Read the model definition and answer for the solid it produces. Units are mm, in the model's axes. Face numbers are marked on the shaded views. Round coordinates to 2 decimals unless told otherwise and drop trailing zeros. Order: outer loops, then holes, each group sorted by start corner. A loop starts at its lowest first (then second) coordinate and runs counter-clockwise, first axis right, second up. Notation, with made-up numbers: (58.5, -10.75) -> (90.5, -10.75) arc R25 cw to (90.5, 26.25) -> close; hole circle Ø1 at (28, 8). An arc over 180 degrees is marked (long way). Answer as a JSON object with one key per item and string values. Group by question number.
Item 1: Given P1, Ø6.5, axis at x = -44, z = -1.5, coming from the +Y side; P2, Ø2, axis at x = -4, z = -8, coming from the +Y side; P3, Ø2, axis at y = -2, z = -8.5, coming from the +X side; P4, Ø4.5, axis at x = -45.5, z = 0, coming from the +Y side, each flat-ended and moving along its own axis, determine where each tip first touches the part or whether it passes through.
Item 2: Section A-A, the plane z = 0 is taken. Count the separate pieces of the cut face and the enclosed holes in it, plus the area to 3 significant figures.
Item 3: Section C-C, the plane z = 10 is taken. Write down the section's boundary in (x, y), plus the area to 3 significant figures.
Item 4: Consider probe 1 along X at (y, z) = (-1.15, 0); probe 2 along Z at (x, y) = (32.5, 1.1); probe 3 along X at (y, z) = (-2.05, 1). Determine where each line is inside the solid, lowest interval first. Write a range as from..to.
Item 5: Section B-B, the plane x = -32 is taken. Write down the section's boundary in (y, z), plus the area to 3 significant figures.
Item 6: The mould has two halves that part along Z. Classify the marked faces 1 and 2: pulls with the +Z half, pulls with the -Z half, needs draft (parallel to the pull), parting line crosses it, or undercut.
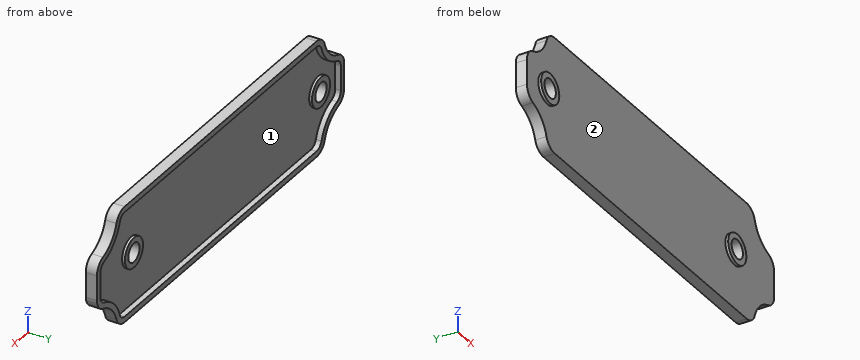
from build123d import *

# Parameters (mm, degrees)
BASE_PLATE_DEPTH                = 1.5
TOP_RECESS_1_5MM_DEPTH          = 1.5
MOUNTING_HOLE_BOSSES_DEPTH      = 0.75
MOUNTING_HOLE_BOSSES_DEPTH_BACK = 2.25
HOLE_BOSS_SKETCH_R              = 4
HOLE_BOSS_SKETCH_R_2            = 2.5
MOUNTING_HOLE_SKETCH_R          = 2.5
MOUNTING_HOLES_2X_DEPTH         = 30.75


with BuildPart() as part:
    # Plate Outline Sketch → Base Plate (new, symmetric)
    with BuildSketch(Plane(origin=(0, 0, 0), x_dir=(1, 0, 0), z_dir=(0, 1, 0))):
        with BuildLine():
            Line((-42.313942393, 15.5), (42.313942393, 15.5))
            ThreePointArc((42.313942393, 15.5), (44.541774365, 14.76649875), (45.898076983, 12.852941176))
            ThreePointArc((45.898076983, 12.852941176), (48.136038969, 9.136038969), (51.852941176, 6.898076983))
            ThreePointArc((51.852941176, 6.898076983), (53.76649875, 5.541774365), (54.5, 3.313942393))
            Line((54.5, 3.313942393), (54.5, -3.313942393))
            ThreePointArc((54.5, -3.313942393), (53.76649875, -5.541774365), (51.852941176, -6.898076983))
            ThreePointArc((51.852941176, -6.898076983), (48.136038969, -9.136038969), (45.898076983, -12.852941176))
            ThreePointArc((45.898076983, -12.852941176), (44.541774365, -14.76649875), (42.313942393, -15.5))
            Line((42.313942393, -15.5), (-42.313942393, -15.5))
            ThreePointArc((-42.313942393, -15.5), (-44.541774365, -14.76649875), (-45.898076983, -12.852941176))
            ThreePointArc((-45.898076983, -12.852941176), (-48.136038969, -9.136038969), (-51.852941176, -6.898076983))
            ThreePointArc((-51.852941176, -6.898076983), (-53.76649875, -5.541774365), (-54.5, -3.313942393))
            Line((-54.5, -3.313942393), (-54.5, 3.313942393))
            ThreePointArc((-54.5, 3.313942393), (-53.76649875, 5.541774365), (-51.852941176, 6.898076983))
            ThreePointArc((-51.852941176, 6.898076983), (-48.136038969, 9.136038969), (-45.898076983, 12.852941176))
            ThreePointArc((-45.898076983, 12.852941176), (-44.541774365, 14.76649875), (-42.313942393, 15.5))
        make_face()
    extrude(amount=BASE_PLATE_DEPTH, both=True)

    # Recess Outline Sketch → Top Recess 1.5mm (cut)
    with BuildSketch(Plane(origin=(0, 1.5, 0), x_dir=(1, 0, 0), z_dir=(0, 1, 0))):
        with BuildLine():
            Line((42.313942393, 14), (-42.313942393, 14))
            ThreePointArc((-42.313942393, 14), (-43.650641576, 13.55989925), (-44.464423147, 12.411764706))
            ThreePointArc((-44.464423147, 12.411764706), (-47.075378798, 8.075378798), (-51.411764706, 5.464423147))
            ThreePointArc((-51.411764706, 5.464423147), (-52.55989925, 4.650641576), (-53, 3.313942393))
            Line((-53, 3.313942393), (-53, -3.313942393))
            ThreePointArc((-53, -3.313942393), (-52.55989925, -4.650641576), (-51.411764706, -5.464423147))
            ThreePointArc((-51.411764706, -5.464423147), (-47.075378798, -8.075378798), (-44.464423147, -12.411764706))
            ThreePointArc((-44.464423147, -12.411764706), (-43.650641576, -13.55989925), (-42.313942393, -14))
            Line((-42.313942393, -14), (42.313942393, -14))
            ThreePointArc((42.313942393, -14), (43.650641576, -13.55989925), (44.464423147, -12.411764706))
            ThreePointArc((44.464423147, -12.411764706), (47.075378798, -8.075378798), (51.411764706, -5.464423147))
            ThreePointArc((51.411764706, -5.464423147), (52.55989925, -4.650641576), (53, -3.313942393))
            Line((53, -3.313942393), (53, 3.313942393))
            ThreePointArc((53, 3.313942393), (52.55989925, 4.650641576), (51.411764706, 5.464423147))
            ThreePointArc((51.411764706, 5.464423147), (47.075378798, 8.075378798), (44.464423147, 12.411764706))
            ThreePointArc((44.464423147, 12.411764706), (43.650641576, 13.55989925), (42.313942393, 14))
        make_face()
    extrude(amount=-TOP_RECESS_1_5MM_DEPTH, mode=Mode.SUBTRACT)

    # Hole Boss Sketch → Mounting Hole Bosses (add, two sides: drawn at the far end of the back side and taken through both)
    # profile 1 of 2: a face of its own
    with BuildSketch(Plane(origin=(0, 0, 0), x_dir=(1, 0, 0), z_dir=(0, 1, 0)).offset(-MOUNTING_HOLE_BOSSES_DEPTH_BACK)):
        with Locations(Location((-45.5, 0, 0), (0, 0, 270))):
            Circle(HOLE_BOSS_SKETCH_R)
        with Locations(Location((-45.5, 0, 0), (0, 0, 270))):
            Circle(HOLE_BOSS_SKETCH_R_2, mode=Mode.SUBTRACT)
    # profile 2 of 2: a face of its own
    with BuildSketch(Plane(origin=(0, 0, 0), x_dir=(1, 0, 0), z_dir=(0, 1, 0)).offset(-MOUNTING_HOLE_BOSSES_DEPTH_BACK)):
        with Locations(Location((36.963444552, -0.123211482, 0), (0, 0, 270))):
            Circle(HOLE_BOSS_SKETCH_R)
        with Locations(Location((36.963444552, -0.123211482, 0), (0, 0, 270))):
            Circle(HOLE_BOSS_SKETCH_R_2, mode=Mode.SUBTRACT)
    extrude(amount=MOUNTING_HOLE_BOSSES_DEPTH + MOUNTING_HOLE_BOSSES_DEPTH_BACK)

    # Mounting Hole Sketch → Mounting Holes 2x (cut)
    with BuildSketch(Plane(origin=(0, 0, 0), x_dir=(1, 0, 0), z_dir=(0, 1, 0))):
        with Locations(Location((36.963444552, -0.123211482, 0), (0, 0, 270))):
            Circle(MOUNTING_HOLE_SKETCH_R)
        with Locations(Location((-45.5, 0, 0), (0, 0, 270))):
            Circle(MOUNTING_HOLE_SKETCH_R)
    extrude(amount=-MOUNTING_HOLES_2X_DEPTH, mode=Mode.SUBTRACT)


solid = part.part
Values found:
{
 "1": {"P1": "y = 0.75", "P2": "y = 0", "P3": "x = 50.13", "P4": "through"},
 "2": {"separate pieces": "3", "enclosed holes": "0", "area": "162 mm2"},
 "3": {"outline": "(-47.38, -1.5) -> (47.38, -1.5) -> (47.38, 1.5) -> (45.56, 1.5) -> (45.56, 0) -> (-45.56, 0) -> (-45.56, 1.5) -> (-47.38, 1.5) -> close", "area": "148 mm2"},
 "4": {"probe 1": "-54.5..-48, -43..34.47, 39.46..54.5", "probe 2": "-15.5..-14, 14..15.5", "probe 3": "-49.37..-47.79, -43.21..-41.63, 33.06..34.62, 39.3..40.87"},
 "5": {"outline": "(-1.5, -15.5) -> (1.5, -15.5) -> (1.5, -14) -> (0, -14) -> (0, 14) -> (1.5, 14) -> (1.5, 15.5) -> (-1.5, 15.5) -> close", "area": "51.0 mm2"},
 "6": {"face 1": "undercut", "face 2": "needs draft"}
}
